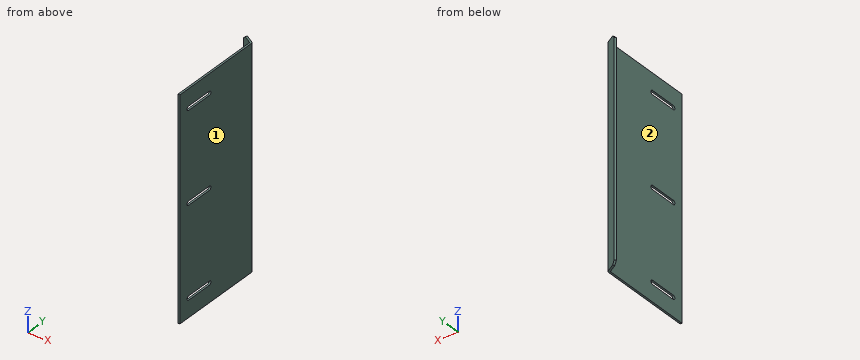
```python
from build123d import *

# Parameters (mm, degrees)
EXTRUDE_1_DEPTH     = 350
CUT_EXTRUDE_1_DEPTH = 382.182371051
CUT_EXTRUDE_2_DEPTH = 382.182371051
CUT_EXTRUDE_3_DEPTH = 382.330464359
CHAMFER_1_SIZE      = 5
FILLET_1_R          = 0.2
FILLET_2_R          = 3.2


with BuildPart() as part:
    # 草图1 → 凸台-拉伸1 (new body)
    with BuildSketch(Plane.XY.offset(350)):
        Polygon((3, -150), (3, 1.732050808), (-15.820508076, 12.598076211), (-17.320508076, 10), (0, 0), (0, -150), align=None)
    extrude(amount=-EXTRUDE_1_DEPTH)

    # 草图2 → 切除-拉伸1 (cut, through all)
    with BuildSketch(Plane.ZY):
        with BuildLine():
            Line((316.75, -88.25), (316.75, -131.75))
            ThreePointArc((316.75, -131.75), (320, -135), (323.25, -131.75))
            Line((323.25, -131.75), (323.25, -88.25))
            ThreePointArc((323.25, -88.25), (320, -85), (316.75, -88.25))
        make_face()
    extrude(amount=-CUT_EXTRUDE_1_DEPTH, mode=Mode.SUBTRACT)

    # 草图3 → 切除-拉伸2 (cut, through all)
    with BuildSketch(Plane.ZY):
        with BuildLine():
            Line((26.75, -88.25), (26.75, -131.75))
            ThreePointArc((26.75, -131.75), (30, -135), (33.25, -131.75))
            Line((33.25, -131.75), (33.25, -88.25))
            ThreePointArc((33.25, -88.25), (30, -85), (26.75, -88.25))
        make_face()
    extrude(amount=-CUT_EXTRUDE_2_DEPTH, mode=Mode.SUBTRACT)

    # 草图4 → 切除-拉伸3 (cut, through all)
    with BuildSketch(Plane(origin=(3, 0, 0), x_dir=(0, 0, -1), z_dir=(1, 0, 0))):
        with BuildLine():
            Line((-171.75, -131.75), (-171.75, -88.25))
            ThreePointArc((-171.75, -88.25), (-175, -85), (-178.25, -88.25))
            Line((-178.25, -88.25), (-178.25, -131.75))
            ThreePointArc((-178.25, -131.75), (-175, -135), (-171.75, -131.75))
        make_face()
    extrude(amount=-CUT_EXTRUDE_3_DEPTH, mode=Mode.SUBTRACT)

    # 倒角1
    chamfer_1_edges = [part.edges().sort_by_distance(p)[0] for p in [
        (-16.570508076, 11.299038106, 0),
        (-16.570508076, 11.299038106, 350),
    ]]
    chamfer(chamfer_1_edges, length=CHAMFER_1_SIZE)

    # 圆角1
    fillet_1_edges = [part.edges().sort_by_distance(p)[0] for p in [
        (0, 0, 175),
    ]]
    fillet(fillet_1_edges, radius=FILLET_1_R)

    # 圆角2
    fillet_2_edges = [part.edges().sort_by_distance(p)[0] for p in [
        (3, 1.732050808, 175),
    ]]
    fillet(fillet_2_edges, radius=FILLET_2_R)


solid = part.part
```
Here's how the part is built. I have some questions about the finished solid (model axes, mm). Face numbers are marked on the shaded views. A direction names the side the tool comes from. Round coordinates to 2 decimals unless told otherwise and drop trailing zeros. Loops run counter-clockwise (first coordinate to the right, second up) from the corner with the lowest first, then second, coordinate; pieces in that order, holes last. Notation, with made-up numbers: (2, 26.25) -> (21, 26.25) arc R16 ccw to (21, 37.25) -> close; hole circle Ø7 at (38, 46). An arc over 180 degrees is marked (long way). Answer as CSV lines item,"result". Start each with the question number.
1. Imagine slicing it at C-C on z = 115. Write out the boundary of the cut face in (x, y).
2. I need wall thicknesses on probe 1 along Z at (x, y) = (1.75, -122); probe 2 along X at (y, z) = (-113.5, 212); probe 3 along Y at (x, z) = (-9.5, 253). Which ranges of each line are inside material? Lowest first, please. Write a range as from..to.
3. For the marked faces 1 and 2, which set-ups out of +Z, -Z, +X, -X, +Y, -Y let a thin tool reach every point of the face, with its end or its side?
4. I'm going to push flat-ended pins straight in: P1, Ø1, axis at x = -6, z = 212, coming from the -Y side; P2, Ø12, axis at x = -6.5, z = 152.5, coming from the -Y side; P3, Ø5, axis at y = -82, z = 182.5, coming from the -X side. Where does each tip first touch, or does it pass through?
5. Imagine slicing it at B-B on z = 30. Write out the boundary of the cut face in (x, y).
6. Imagine slicing it at D-D on y = -70. Write out the boundary of the cut face in (x, z), plus the area to 3 significant figures.
7. Imagine slicing it at A-A on y = -112.5. Write out the boundary of the cut face in (x, z), plus the area to 4 significant figures.
Solution:
1,outline,"(-17.32, 10) -> (-0.1, 0.06) arc R0.2 cw to (0, -0.12) -> (0, -150) -> (3, -150) -> (3, -0.12) arc R3.2 ccw to (1.4, 2.66) -> (-15.82, 12.6) -> close"
2,probe 1,"0..26.75, 33.25..171.75, 178.25..316.75, 323.25..350"
2,probe 2,"0..3"
2,probe 3,"5.48..8.95"
3,face 1,"+Z, -Z, +X, +Y, -Y"
3,face 2,"+Z, -Z, -X, -Y"
4,P1,"y = 3.18"
4,P2,"y = 0.29"
4,P3,"x = 0"
5,outline,"(-17.32, 10) -> (-0.1, 0.06) arc R0.2 cw to (0, -0.12) -> (0, -85) -> (3, -85) -> (3, -0.12) arc R3.2 ccw to (1.4, 2.66) -> (-15.82, 12.6) -> close; (0, -150) -> (3, -150) -> (3, -135) -> (0, -135) -> close"
6,outline,"(0, 0) -> (3, 0) -> (3, 350) -> (0, 350) -> close"
6,area,"1,050 mm²"
7,outline,"(0, 0) -> (3, 0) -> (3, 26.75) -> (0, 26.75) -> close; (0, 33.25) -> (3, 33.25) -> (3, 171.75) -> (0, 171.75) -> close; (0, 178.25) -> (3, 178.25) -> (3, 316.75) -> (0, 316.75) -> close; (0, 323.25) -> (3, 323.25) -> (3, 350) -> (0, 350) -> close"
7,area,"991.5 mm²"
